For this review, use the dimensioned drawing (mm, ordinates from the lowest corner) and the shaded views. Coordinates: 2 decimals unless noted, no trailing zeros. Write each loop counter-clockwise with the first axis right and the second up, starting at its lowest first coordinate (ties: lowest second). Pieces come first, ordered by that corner, then holes. Notation, with made-up numbers: (26, -26) - (80, -26) arc R24 cw to (80, 5) - close; hole circle Ø8 at (49.25, 49.5). An arc over 180 degrees is marked (long way). Use one line per item in the form item = value. Start each with the question number.
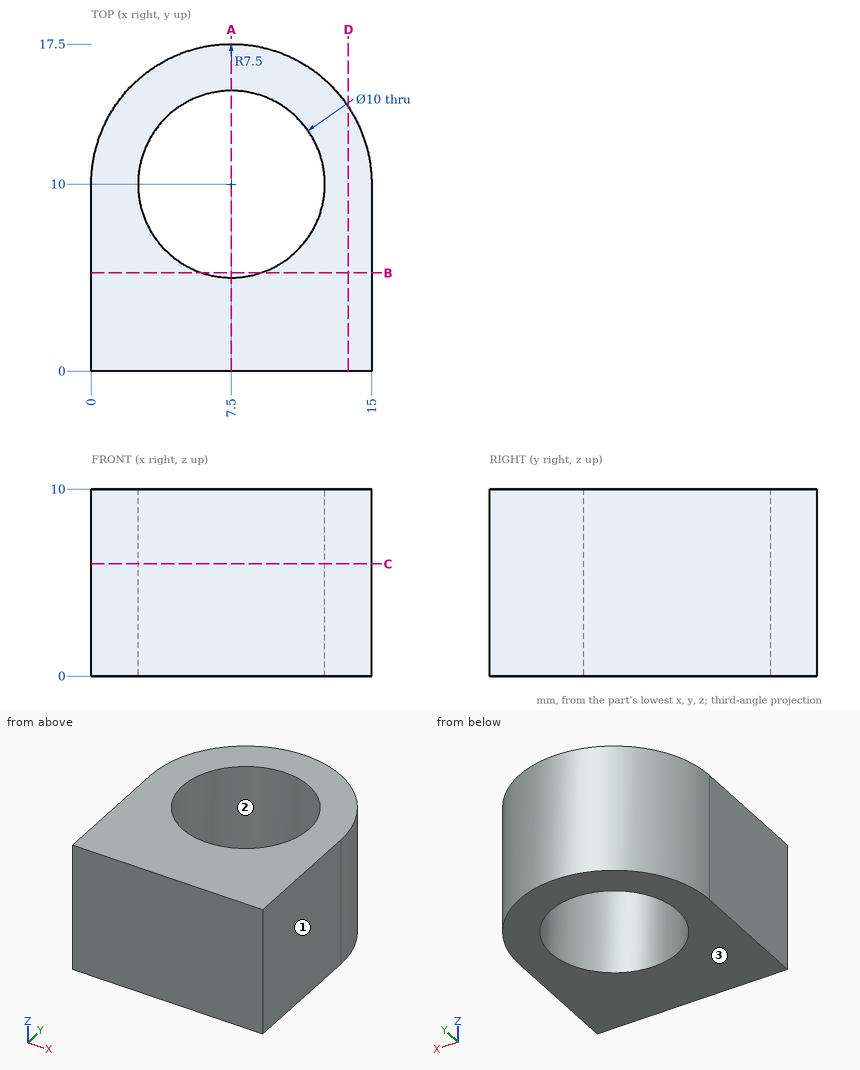
1. For L1, parallel to Y at x = 7.5, z = 6.75; L2, parallel to X at y = 9.75, z = 4; L3, parallel to Y at x = 6.5, z = 2, list the stretches that pass through material, from the lowest coordinate up.
2. For P1, Ø1.5, axis at y = 12.5, z = 2.5, coming from the +X side, flat-tipped, find the tip position at first contact; note if it passes through.
3. The part is to be moulded in two halves that separate along X. For the marked faces 1, 2 and 3, say which applies: released by +X, released by -X, zero draft, split by the parting line, or undercut.
4. Take a section at D-D (x = 13.75). State the section outline as (y, z) points, plus the area to 3 significant figures.
5. Take a section at A-A (x = 7.5). State the section outline as (y, z) points, plus the area to 3 significant figures.
6. Take a section at B-B (y = 5.25). State the section outline as (x, z) points, plus the area to 3 significant figures.
7. Take a section at C-C (z = 6). State the section outline as (x, y) points, plus the area to 3 significant figures.
Returned:
q1.L1 = 0 to 5, 15 to 17.5
q1.L2 = 0 to 2.51, 12.49 to 15
q1.L3 = 0 to 5.1, 14.9 to 17.43
q2.P1 = 14.79
q3.face_1 = released by +X
q3.face_2 = undercut
q3.face_3 = zero draft
q4.outline = (0, 0) - (14.15, 0) - (14.15, 10) - (0, 10) - close
q4.area = 141 mm²
q5.outline = (0, 0) - (5, 0) - (5, 10) - (0, 10) - close; (15, 0) - (17.5, 0) - (17.5, 10) - (15, 10) - close
q5.area = 75.0 mm²
q6.outline = (0, 0) - (5.94, 0) - (5.94, 10) - (0, 10) - close; (9.06, 0) - (15, 0) - (15, 10) - (9.06, 10) - close
q6.area = 119 mm²
q7.outline = (0, 0) - (15, 0) - (15, 10) arc R7.5 ccw to (0, 10) - close; hole circle Ø10 at (7.5, 10)
q7.area = 160 mm²
